For this review, take the finished solid that the model builds, in its own axes (mm). A direction names the side the tool comes from. Give positions to 0.01 mm unless a question says otherwise; leave off trailing zeros. Loops run counter-clockwise (first coordinate to the right, second up) from the corner with the lowest first, then second, coordinate; pieces in that order, holes last. Notation, with made-up numbers: (41.25, 28.5) - (84.25, 28.5) arc R12 ccw to (84.25, 40.5) - close; hole circle Ø1 at (-2, 73.5). An arc over 180 degrees is marked (long way). Use CSV: the item, a comma, the result in double quotes. Start each with the question number.
1. Take a section at C-C on y = -32.5. Give the boundary of the cut face in (x, z).
2. Take a section at A-A on z = 0. Give the boundary of the cut face in (x, y), plus the area to 3 significant figures.
3. For pin 1 (10 mm diameter, centred on x = -13, y = 15, fed in from -Z); pin 2 (12 mm diameter, centred on x = 17, y = -0.5, fed in from -Z); pin 3 (5 mm diameter, centred on x = 21, y = -0.5, fed in from +Z), all flat-tipped, find the tip position at first contact; note any pin that passes through.
4. Take a section at B-B on x = 24.5. Give the boundary of the cut face in (y, z), plus the area to 3 significant figures.
5. Wall thickness on line 1 (Y direction, x = 49, z = 10); line 2 (X direction, y = 27.5, z = 6); line 3 (X direction, y = 1, z = -8.5): over which ranges is each line inside the solid? List them lowest first.
6. For faces 1 (the flat face through (12, -7, 0)), 2 (the flat face through (-23, -13, -33)), 3 (the cylindrical face through (-0.322, -45.445, -12.015)), list the 3-axis set-ups (+Z, -Z, +X, -X, +Y, -Y) from which the entire face can be reached by the end or side of a thin tool; tool diameter is ignored.
7. Take a section at D-D on x = 1.5. Give the boundary of the cut face in (y, z).
8. Mouldability with a two-part tool opening along Y and no side actions: class faces 4 (the cylindrical face through (34.82, -18.4, -8.52)), 5 (the flat face through (57, 7, 0)), 6 (the cylindrical face through (39.762, -0.138, 32.215)) as pulls with the +Y half, pulls with the -Y half, needs draft (parallel to the pull), parting line crosses it, or undercut.
```python
from build123d import *

# Parameters (mm, degrees)
SKETCH_2_R          = 11
CUT_EXTRUDE_1_DEPTH = 45
SKETCH_3_R          = 14
CUT_EXTRUDE_2_DEPTH = 45


with BuildPart() as part:
    # 草图1 → 旋转1 (revolve)
    with BuildSketch(Plane.XY, mode=Mode.PRIVATE) as revolve_1_sk:
        Polygon((-57, -7.291938998), (57, -7.291938998), (57, 25.708061002), (23, 25.708061002), (23, 32.708061002), (-23, 32.708061002), (-23, 25.708061002), (-57, 25.708061002), align=None)
    revolve(revolve_1_sk.sketch.rotate(Axis((-57, -7.291938998, 0), (1, 0, 0)), 180), axis=Axis((-57, -7.291938998, 0), (1, 0, 0)))

    # 草图2 → 切除-拉伸1 (cut)
    with BuildSketch(Plane.ZY.offset(57)):
        with Locations(Location((0, -7.291938998, 0), (0, 0, 270))):
            Circle(SKETCH_2_R)
    extrude(amount=-CUT_EXTRUDE_1_DEPTH, mode=Mode.SUBTRACT)

    # 草图3 → 切除-拉伸2 (cut)
    with BuildSketch(Plane(origin=(57, 0, 0), x_dir=(0, 0, -1), z_dir=(1, 0, 0))):
        with Locations(Location((0, -7.291938998, 0), (0, 0, 90))):
            Circle(SKETCH_3_R)
    extrude(amount=-CUT_EXTRUDE_2_DEPTH, mode=Mode.SUBTRACT)


solid = part.part
```
Check result:
1,outline,"(-57, -21.3) - (-23, -21.3) - (-23, -31.06) - (23, -31.06) - (23, -21.3) - (57, -21.3) - (57, 21.3) - (23, 21.3) - (23, 31.06) - (-23, 31.06) - (-23, 21.3) - (-57, 21.3) - close"
2,outline,"(-57, -40.29) - (-23, -40.29) - (-23, -47.29) - (23, -47.29) - (23, -40.29) - (57, -40.29) - (57, -21.29) - (12, -21.29) - (12, 6.71) - (57, 6.71) - (57, 25.71) - (23, 25.71) - (23, 32.71) - (-23, 32.71) - (-23, 25.71) - (-57, 25.71) - (-57, 3.71) - (-12, 3.71) - (-12, -18.29) - (-57, -18.29) - close"
2,area,"5,920 mm²"
3,pin 1,"stops at z = -36.07"
3,pin 2,"stops at z = -39.99"
3,pin 3,"stops at z = 39.77"
4,outline,"circle Ø66 at (-7.29, 0); hole circle Ø28 at (-7.29, 0)"
4,area,"2,810 mm²"
5,line 1,"y = -38.74 to -17.09, 2.51 to 24.16"
5,line 2,"x = -23 to 23"
5,line 3,"x = -57 to 12"
6,face 1,"+X"
6,face 2,"-X"
6,face 3,"+X, -X"
7,outline,"circle Ø80 at (-7.29, 0)"
8,face 4,"undercut"
8,face 5,"needs draft"
8,face 6,"parting line crosses it"
